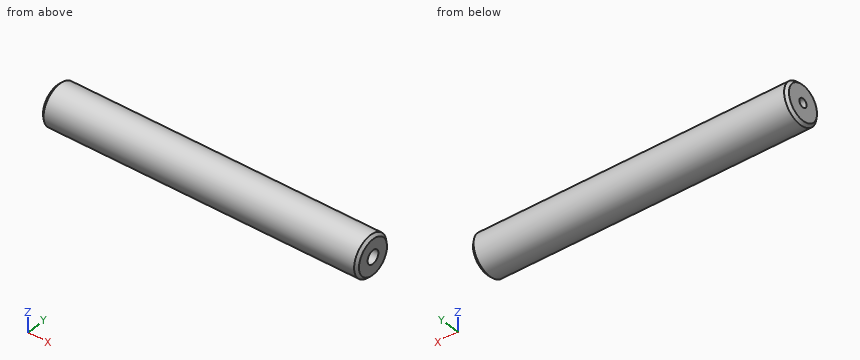
```python
from build123d import *

# Parameters (mm, degrees)
SKETCH_1_R             = 7.5
EXTRUDE_1_DEPTH        = 117
HOLE_WIZARD_M4_1_D     = 3.3
HOLE_WIZARD_M4_1_DEPTH = 10.1
HOLE_WIZARD_M4_1_TIP   = 0.991420021
HOLE_WIZARD_M6_1_D     = 5
HOLE_WIZARD_M6_1_DEPTH = 15
HOLE_WIZARD_M6_1_TIP   = 1.502151548
CHAMFER_1_SIZE         = 1


with BuildPart() as part:
    # 草图1 → 凸台-拉伸1 (new body)
    with BuildSketch(Plane(origin=(0, 0, 0), x_dir=(0, 0, -1), z_dir=(1, 0, 0))):
        Circle(SKETCH_1_R)
    extrude(amount=EXTRUDE_1_DEPTH)

    # M4 螺纹孔1
    with Locations(Plane.ZY):
        with Locations((0, 0)):
            Hole(HOLE_WIZARD_M4_1_D / 2, depth=HOLE_WIZARD_M4_1_DEPTH)
            with Locations((0, 0, -(HOLE_WIZARD_M4_1_DEPTH + HOLE_WIZARD_M4_1_TIP / 2))):  # 118° drill point
                Cone(0, HOLE_WIZARD_M4_1_D / 2, HOLE_WIZARD_M4_1_TIP, mode=Mode.SUBTRACT)

    # M6 螺纹孔1
    with Locations(Plane(origin=(117, 0, 0), x_dir=(0, 0, -1), z_dir=(1, 0, 0))):
        with Locations((0, 0)):
            Hole(HOLE_WIZARD_M6_1_D / 2, depth=HOLE_WIZARD_M6_1_DEPTH)
            with Locations((0, 0, -(HOLE_WIZARD_M6_1_DEPTH + HOLE_WIZARD_M6_1_TIP / 2))):  # 118° drill point
                Cone(0, HOLE_WIZARD_M6_1_D / 2, HOLE_WIZARD_M6_1_TIP, mode=Mode.SUBTRACT)

    # 倒角1
    chamfer_1_edges = [part.edges().sort_by_distance(p)[0] for p in [
        (0, 0, 7.5),
        (117, 0, 7.5),
    ]]
    chamfer(chamfer_1_edges, length=CHAMFER_1_SIZE)


solid = part.part
```
Build history of the part. All positions in model axes, mm. Coordinates: 2 decimals unless noted, no trailing zeros. Order: outer loops, then holes, each group sorted by start corner. A loop starts at its lowest first (then second) coordinate and runs counter-clockwise, first axis right, second up.
Item 1: Drill centre lines: L1, parallel to Y at x = 107, z = 0; L2, parallel to Y at x = 2.75, z = 0; L3, parallel to X at y = 3.5, z = 5.5. Where is each one in solid material? Low to high.
Filled in:
L1: y = -7.5 to -2.5, 2.5 to 7.5
L2: y = -7.5 to -1.65, 1.65 to 7.5
L3: x = 0.02 to 116.98
Item 2: Drop flat-ended pins along their axis: pin 1 Ø4 at (y, z) = (0, 0) entering from +X; pin 2 Ø1 at (x, y) = (63.5, 5.5) entering from -Z; pin 3 Ø3 at (y, z) = (0, 0) entering from -X. Give the stop position or say it passes through.
Filled in:
pin 1: stops at x = 101.7
pin 2: stops at z = -5.59
pin 3: stops at x = 10.19
Item 3: Saw through at A-A on x = 61.5. List the corners of the cut face in (y, z).
Filled in:
outline: circle Ø15 at (0, 0)
